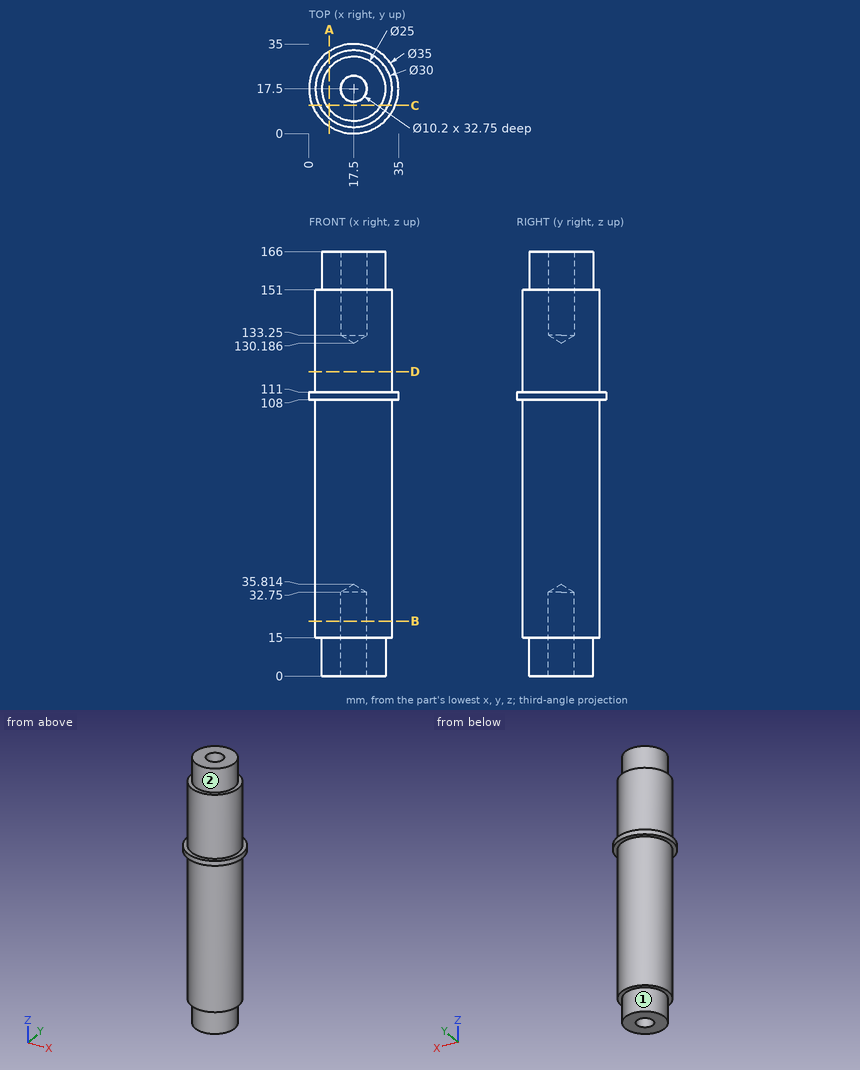
Here's the drawing with two shaded views (mm, measured from the low corner). I have some questions. A direction names the side the tool comes from. Give positions to 0.01 mm unless a question says otherwise; leave off trailing zeros. Loops run counter-clockwise (first coordinate to the right, second up) from the corner with the lowest first, then second, coordinate; pieces in that order, holes last. Notation, with made-up numbers: (52.5, 53) - (57.5, 53) arc R14 ccw to (57.5, 66) - close; hole circle Ø6 at (77, 56.25). An arc over 180 degrees is marked (long way). Answer in a Markdown table with one row per item. Add a question column.
Q1. Which directions (+Z, -Z, +X, -X, +Y, -Y) give clear straight access to the entire face, cutting with the end or side of a thin tool? Please do the marked faces 1 and 2.
Q2. Please list where these lines run through material, in increasing order: L1, parallel to Y at x = 17.5, z = 144.5; L2, parallel to Y at x = 17, z = 9 (1 decimal). Write a range as from..to.
Q3. If we section it at B-B (z = 21.5): List the corners of the cut face in (x, y) for me, plus the area to 3 significant figures.
Q4. If we section it at D-D (z = 119): List the corners of the cut face in (x, y) for me.
Q5. For pin 1 (8 mm diameter, centred on x = 18.5, y = 10.5, fed in from -Z); pin 2 (10 mm diameter, centred on x = 21.5, z = 44.5, fed in from +Y); pin 3 (4 mm diameter, centred on x = 18.5, z = 128, fed in from -Y); pin 4 (5 mm diameter, centred on x = 27.5, z = 128.5, fed in from +Y), each with a flat end and sliding along its axis, tell me the tip position at first contact or that it passes through.
Q6. If we section it at C-C (y = 11): List the corners of the cut face in (x, z) for me.
Q7. If we section it at A-A (x = 8): List the corners of the cut face in (y, z) for me, plus the area to 3 significant figures.
The answers:
| question | item | result |
|---|---|---|
| 1 | face 1 | -Z |
| 1 | face 2 | +Z |
| 2 | L1 | y = 2.5..12.4, 22.6..32.5 |
| 2 | L2 | y = 5..12.4, 22.6..30 |
| 3 | outline | circle Ø30 at (17.5, 17.5); hole circle Ø10.2 at (17.5, 17.5) |
| 3 | area | 625 mm^2 |
| 4 | outline | circle Ø30 at (17.5, 17.5) |
| 5 | pin 1 | stops at z = 0 |
| 5 | pin 2 | stops at y = 32.5 |
| 5 | pin 3 | stops at y = 2.5 |
| 5 | pin 4 | stops at y = 30.49 |
| 6 | outline | (1.25, 108) - (3.98, 108) - (3.98, 15) - (6.82, 15) - (6.82, 0) - (28.18, 0) - (28.18, 15) - (31.02, 15) - (31.02, 108) - (33.75, 108) - (33.75, 111) - (31.02, 111) - (31.02, 151) - (28.18, 151) - (28.18, 166) - (6.82, 166) - (6.82, 151) - (3.98, 151) - (3.98, 111) - (1.25, 111) - close |
| 7 | outline | (2.8, 108) - (5.89, 108) - (5.89, 15) - (9.38, 15) - (9.38, 0) - (25.62, 0) - (25.62, 15) - (29.11, 15) - (29.11, 108) - (32.2, 108) - (32.2, 111) - (29.11, 111) - (29.11, 151) - (25.62, 151) - (25.62, 166) - (9.38, 166) - (9.38, 151) - (5.89, 151) - (5.89, 111) - (2.8, 111) - close |
| 7 | area | 3,660 mm^2 |
